Job drawing, mm, ordinate dimensions from the low corner. One solid piece. A direction names the side the tool comes from. Round coordinates to 2 decimals unless told otherwise and drop trailing zeros. Write each loop counter-clockwise with the first axis right and the second up, starting at its lowest first coordinate (ties: lowest second). Pieces come first, ordered by that corner, then holes.
1) Pull direction X, two halves, no side cores. Call the marked faces 1, 2, 3 and 4: +X half, -X half, draft (parallel to the pull), parting line (faces both ways), or undercut.
2) Wall check: probe 1 along X at (y, z) = (24, 21); probe 2 along Z at (x, y) = (80, 27); probe 3 along X at (y, z) = (21, 16). Give the ranges that are in metal, low to high.
3) Saw through at A-A (z = 21). Write the cut outline in (x, y), plus the area to 3 significant figures.
4) Saw through at B-B (y = 18.5). Write the cut outline in (x, z), plus the area to 3 significant figures.
5) Saw through at D-D (y = 31). Write the cut outline in (x, z).
6) Saw through at C-C (x = 27.5). Write the cut outline in (y, z).
7) Which spindle directions (+Z, -Z, +X, -X, +Y, -Y) get a long thin tool onto all of the face, cutting with end or side? Do the marked faces 5 and 6. Say none if no direction does.
8) Flat gauge pins, fed straight in: pin 1 (10.5 mm diameter, centred on x = 35.5, y = 10, fed in from +Z); pin 2 (1.5 mm diameter, centred on y = 13.5, z = 9.5, fed in from +X); pin 3 (6 mm diameter, centred on x = 69, y = 28, fed in from +Z); pin 4 (1 mm diameter, centred on x = 74, z = 29, fed in from -Y). Where does each tip first touch, or does it go through?
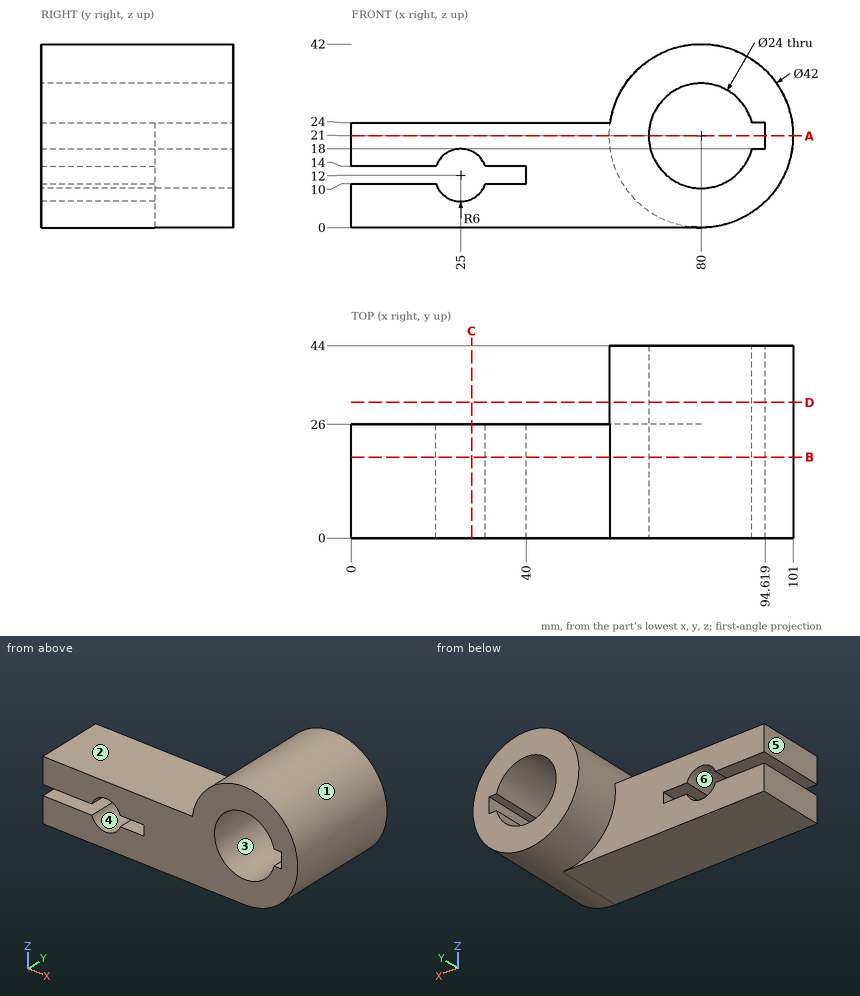
Evaluation:
1. face 1: parting line
1. face 2: draft
1. face 3: undercut
1. face 4: undercut
2. probe 1: x = 0 to 68, 94.62 to 101
2. probe 2: z = 0 to 9, 33 to 42
2. probe 3: x = 0 to 20.53, 29.47 to 69.09, 90.91 to 100.4
3. outline: (0, 0) - (68, 0) - (68, 44) - (59, 44) - (59, 26) - (0, 26) - close; (94.62, 0) - (101, 0) - (101, 44) - (94.62, 44) - close
3. area: 2,210 mm2
4. outline: (0, 0) - (80, 0) arc R21 ccw (long way) to (59.22, 24) - (0, 24) - (0, 14) - (19.34, 14) arc R6 cw to (30.66, 14) - (40, 14) - (40, 10) - (30.66, 10) arc R6 cw to (19.34, 10) - (0, 10) - close; hole (91.62, 18) - (94.62, 18) - (94.62, 24) - (91.62, 24) arc R12 ccw (long way) to start
4. area: 2,200 mm2
5. outline: circle Ø42 at (80, 21); hole (91.62, 18) - (94.62, 18) - (94.62, 24) - (91.62, 24) arc R12 ccw (long way) to start
6. outline: (0, 0) - (26, 0) - (26, 6.55) - (0, 6.55) - close; (0, 17.45) - (26, 17.45) - (26, 24) - (0, 24) - close
7. face 5: +Z, -Z, -X, +Y, -Y
7. face 6: +Y, -Y
8. pin 1: stops at z = 24
8. pin 2: stops at x = 98.04
8. pin 3: stops at z = 40.42
8. pin 4: passes through
